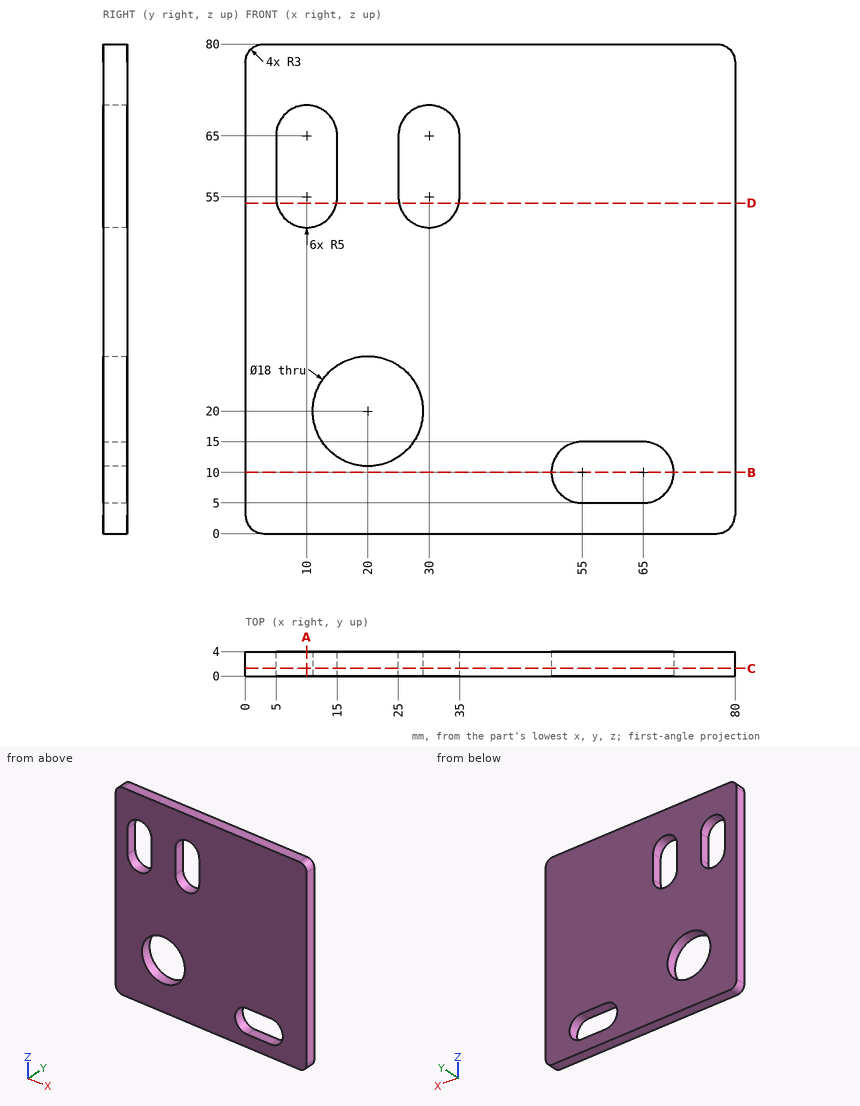
Geometry check sheet. Reference: drawing and pictorial views, mm from the part's lowest x, y, z. Give positions to 0.01 mm unless a question says otherwise; leave off trailing zeros. Write each loop counter-clockwise with the first axis right and the second up, starting at its lowest first coordinate (ties: lowest second). Pieces come first, ordered by that corner, then holes.
Item 1: Cross-section at C-C (y = 1.25). Enter the section's corners in (x, z), and give its area (3 significant figures).
Item 2: Cross-section at D-D (z = 54). Enter the section's corners in (x, y).
Item 3: Cross-section at B-B (z = 10). Enter the section's corners in (x, y), and give its area (3 significant figures).
Item 4: Gauge pin test, flat end, axial feed: pin 1 (20.5 mm diameter, centred on x = 20, z = 20, fed in from +Y). Record the tip position at first contact, or that the pin passes through.
Item 5: Cross-section at A-A (x = 10). Enter the section's corners in (y, z), and give its area (3 significant figures).
Item 6: Scan lines: L1, parallel to X at y = 1.4, z = 57; L2, parallel to Z at x = 55, y = 3.3; L3, parallel to X at y = 1.1, z = 20. Record each from-to range of solid material in increasing order.
Report:
1. outline: (0, 3) arc R3 ccw to (3, 0) - (77, 0) arc R3 ccw to (80, 3) - (80, 77) arc R3 ccw to (77, 80) - (3, 80) arc R3 ccw to (0, 77) - close; hole (5, 55) arc R5 ccw to (15, 55) - (15, 65) arc R5 ccw to (5, 65) - close; hole circle Ø18 at (20, 20); hole (25, 55) arc R5 ccw to (35, 55) - (35, 65) arc R5 ccw to (25, 65) - close; hole (55, 5) - (65, 5) arc R5 ccw to (65, 15) - (55, 15) arc R5 ccw to start
1. area: 5,600 mm2
2. outline: (0, 0) - (5.1, 0) - (5.1, 4) - (0, 4) - close; (14.9, 0) - (25.1, 0) - (25.1, 4) - (14.9, 4) - close; (34.9, 0) - (80, 0) - (80, 4) - (34.9, 4) - close
3. outline: (0, 0) - (50, 0) - (50, 4) - (0, 4) - close; (70, 0) - (80, 0) - (80, 4) - (70, 4) - close
3. area: 240 mm2
4. pin 1: stops at y = 4
5. outline: (0, 0) - (4, 0) - (4, 50) - (0, 50) - close; (0, 70) - (4, 70) - (4, 80) - (0, 80) - close
5. area: 240 mm2
6. L1: x = 0 to 5, 15 to 25, 35 to 80
6. L2: z = 0 to 5, 15 to 80
6. L3: x = 0 to 11, 29 to 80
